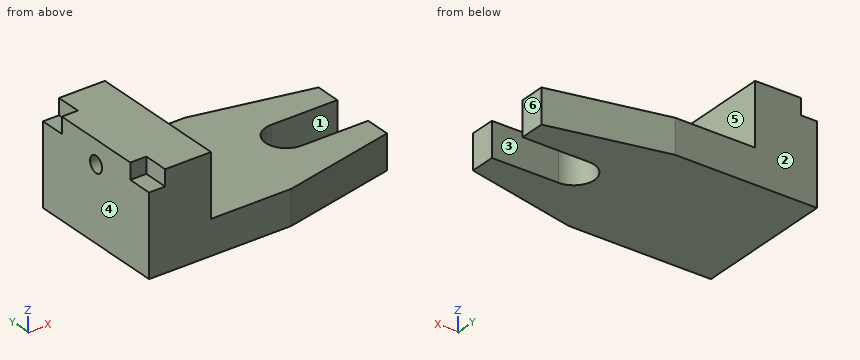
```python
from build123d import *

# Parameters (mm, degrees)
FORK_ARM_PLATE_DEPTH    = 15
MOUNTING_BLOCK_SKETCH_W = 27
MOUNTING_BLOCK_SKETCH_H = 62
MOUNTING_BLOCK_DEPTH    = 42
BLOCK_STEP_CUT_SKETCH_W = 7
BLOCK_STEP_CUT_SKETCH_H = 11
BLOCK_STEP_CUT_DEPTH    = 7
SIDE_HOLE_7_SKETCH_R    = 3.5
SIDE_HOLE_7_DEPTH       = 135.729358345


with BuildPart() as part:
    # Fork Arm Profile Sketch → Fork Arm Plate (new body)
    with BuildSketch(Plane.XY):
        with BuildLine():
            ThreePointArc((56, 40), (47, 31), (56, 22))
            Line((56, 22), (85, 22))
            Line((85, 22), (85, 11))
            Line((85, 11), (35, 0))
            Line((35, 0), (0, 0))
            Line((0, 0), (0, 62))
            Line((0, 62), (35, 62))
            Line((35, 62), (85, 51))
            Line((85, 51), (85, 40))
            Line((85, 40), (56, 40))
        make_face()
    extrude(amount=FORK_ARM_PLATE_DEPTH)

    # Mounting Block Sketch → Mounting Block (add)
    with BuildSketch(Plane.XY):
        with Locations((-13.5, 31)):
            Rectangle(MOUNTING_BLOCK_SKETCH_W, MOUNTING_BLOCK_SKETCH_H)
    extrude(amount=MOUNTING_BLOCK_DEPTH)

    # Block Step Cut Sketch → Block Step Cut (cut)
    with BuildSketch(Plane.ZY.offset(27)):
        with Locations((38.5, 56.5)):
            Rectangle(BLOCK_STEP_CUT_SKETCH_W, BLOCK_STEP_CUT_SKETCH_H)
        with Locations((38.5, 5.5)):
            Rectangle(BLOCK_STEP_CUT_SKETCH_W, BLOCK_STEP_CUT_SKETCH_H)
    extrude(amount=-BLOCK_STEP_CUT_DEPTH, mode=Mode.SUBTRACT)

    # Side Hole Ø7 Sketch → Side Hole Ø7 (cut, through all)
    with BuildSketch(Plane.ZY.offset(27)):
        with Locations((32, 31)):
            Circle(SIDE_HOLE_7_SKETCH_R)
    extrude(amount=-SIDE_HOLE_7_DEPTH, mode=Mode.SUBTRACT)


solid = part.part
```
Geometry: final body of the model. Coordinates: model frame, mm. Face numbers are marked on the shaded views. A direction names the side the tool comes from. Round coordinates to 2 decimals unless told otherwise and drop trailing zeros. Write each loop counter-clockwise with the first axis right and the second up, starting at its lowest first coordinate (ties: lowest second). Pieces come first, ordered by that corner, then holes. Notation, with made-up numbers: M -7,55 L 32,55 A28 cw 32,83 Z; hole C 72.5,20 d10. An arc over 180 degrees is marked long. Answer in a Markdown table with one row per item. Add a question column.
(1) Cut plane A-A, the plane y = 31. Return the cut outline in (x, z), then the cut area to 3 significant figures.
(2) Cut plane D-D, the plane y = 56.5. Return the cut outline in (x, z), then the cut area to 4 significant figures.
(3) Ray query, L1, parallel to Y at x = -21, z = 32; L2, parallel to X at y = 23.5, z = 29; L3, parallel to Z at x = 34.5, y = 54.5. Return the intervals inside material, ascending.
(4) Contact query for flat-ended pins moving along their axis: pin 1 (3.5 mm diameter, centred on y = 55.5, z = 37.5, fed in from -X); pin 2 (4 mm diameter, centred on y = 48.5, z = 35.5, fed in from +X); pin 3 (3.5 mm diameter, centred on x = -23, z = 39, fed in from -Y). Output: stop coordinate, or through.
(5) Reachability of the marked faces 5 and 6 from +Z, -Z, +X, -X, +Y, -Y: full face, straight path, thin tool, end or side. Return the list, or none.
(6) Cut plane B-B, the plane x = 65. Return the cut outline in (y, z).
(7) Cut plane C-C, the plane z = 32. Return the cut outline in (x, y).
(8) Draft query along Y for the marked faces 1, 2, 3 and 4. Return one class per face: pulls with the +Y half, pulls with the -Y half, needs draft (parallel to the pull), parting line crosses it, or undercut.
Established:
| question | item | result |
|---|---|---|
| 1 | outline | M -27,0 L 47,0 L 47,15 L 0,15 L 0,28.5 L -27,28.5 Z; M -27,35.5 L 0,35.5 L 0,42 L -27,42 Z |
| 1 | area | 1,650 mm² |
| 2 | outline | M -27,0 L 60,0 L 60,15 L 0,15 L 0,42 L -20,42 L -20,35 L -27,35 Z |
| 2 | area | 1,985 mm² |
| 3 | L1 | 0 to 27.5, 34.5 to 62 |
| 3 | L2 | -27 to 0 |
| 3 | L3 | 0 to 15 |
| 4 | pin 1 | x = -20 |
| 4 | pin 2 | x = 0 |
| 4 | pin 3 | y = 11 |
| 5 | face 5 | +Z, +X, +Y, -Y |
| 5 | face 6 | +Z, -Z, +X, +Y, -Y |
| 6 | outline | M 6.6,0 L 22,0 L 22,15 L 6.6,15 Z; M 40,0 L 55.4,0 L 55.4,15 L 40,15 Z |
| 7 | outline | M -27,0 L 0,0 L 0,27.5 L -27,27.5 Z; M -27,34.5 L 0,34.5 L 0,62 L -27,62 Z |
| 8 | face 1 | undercut |
| 8 | face 2 | pulls with the +Y half |
| 8 | face 3 | undercut |
| 8 | face 4 | needs draft |
